```python
from build123d import *

# Parameters (mm, degrees)
BOSS_EXTRUDE1_DEPTH = 12


with BuildPart() as part:
    # Sketch1 → Boss-Extrude1 (new body)
    with BuildSketch(Plane.XY):
        with BuildLine():
            Line((140, 147), (378, 147))
            ThreePointArc((378, 147), (406.284271247, 135.284271247), (418, 107))
            Line((418, 107), (418, 0))
            Line((418, 0), (944.5, 0))
            Line((944.5, 0), (958.236494969, 111.874773736))
            ThreePointArc((958.236494969, 111.874773736), (971.433539106, 136.958228832), (997.938341035, 147))
            Line((997.938341035, 147), (1273.561658965, 147))
            ThreePointArc((1273.561658965, 147), (1300.066460894, 136.958228832), (1313.263505031, 111.874773736))
            Line((1313.263505031, 111.874773736), (1327, 0))
            Line((1327, 0), (1843, 0))
            Line((1843, 0), (1843, 107))
            ThreePointArc((1843, 107), (1854.715728753, 135.284271247), (1883, 147))
            Line((1883, 147), (2158, 147))
            ThreePointArc((2158, 147), (2186.284271247, 135.284271247), (2198, 107))
            Line((2198, 107), (2198, 0))
            Line((2198, 0), (2388, 0))
            Line((2388, 0), (2400, 12))
            Line((2400, 12), (2400, 195))
            Line((2400, 195), (2388, 207))
            Line((2388, 207), (12, 207))
            Line((12, 207), (0, 195))
            Line((0, 195), (0, 12))
            Line((0, 12), (12, 0))
            Line((12, 0), (100, 0))
            Line((100, 0), (100, 107))
            ThreePointArc((100, 107), (111.715728753, 135.284271247), (140, 147))
        make_face()
    extrude(amount=BOSS_EXTRUDE1_DEPTH)


solid = part.part
```
CAD build for the part. Positions are in the model's coordinates, mm. A direction names the side the tool comes from. Coordinates: 2 decimals unless noted, no trailing zeros. Loops run counter-clockwise (first coordinate to the right, second up) from the corner with the lowest first, then second, coordinate; pieces in that order, holes last. Notation, with made-up numbers: (23, -37) - (35, -37) arc R6 ccw to (35, -27) - close; hole circle Ø4 at (50.25, -37.5). An arc over 180 degrees is marked (long way). Use CSV: the item, a comma, the result in double quotes. Start each with the question number.
Q1. Drop flat-ended pins along their axis: P1, Ø3, axis at y = 185, z = 4.5, coming from the -X side; P2, Ø3, axis at x = 1288, z = 3.5, coming from the -Y side; P3, Ø6, axis at x = 2037.5, z = 8, coming from the -Y side. Give the stop position or say it passes through.
Q2. Probe probe 1 along X at (y, z) = (111, 4.75); probe 2 along X at (y, z) = (124.5, 3.75); probe 3 along Y at (x, z) = (1896, 11). List the from-to ranges inside material, lowest first. Write a range as from..to.
Q3. Cut at A-A, the plane y = 51. List the corners of the cut face in (x, z).
Q4. Two-plate mould, pull along X, no slides. Class faces 3 (the flat face through (1183, 151, 12)), 4 (the cylindrical face through (1854.406, 134.972, 5.916)): +X half, -X half, draft (parallel to the pull), parting line (faces both ways), or undercut.
Q5. Cut at C-C, the plane x = 270. List the corners of the cut face in (y, z).
Q6. Cut at B-B, the plane z = 2.75. List the corners of the cut face in (x, y).
Q7. 3-axis set-ups, long thin cutter, end or side, ignore diameter. For faces 1 (the flat face through (1183, 151, 0)), 2 (the cylindrical face through (405.972, 135.594, 5.916)): which of +Z, -Z, +X, -X, +Y, -Y reach the whole face in a straight line?
Here are the results:
1,P1,"x = 0"
1,P2,"y = 143.69"
1,P3,"y = 147"
2,probe 1,"0..100.2, 417.8..958.13, 1313.37..1843.2, 2197.8..2400"
2,probe 2,"0..104.03, 413.97..961.97, 1309.53..1847.03, 2193.97..2400"
2,probe 3,"147..207"
3,outline,"(0, 0) - (100, 0) - (100, 12) - (0, 12) - close; (418, 0) - (950.76, 0) - (950.76, 12) - (418, 12) - close; (1320.74, 0) - (1843, 0) - (1843, 12) - (1320.74, 12) - close; (2198, 0) - (2400, 0) - (2400, 12) - (2198, 12) - close"
4,face 3,"draft"
4,face 4,"undercut"
5,outline,"(147, 0) - (207, 0) - (207, 12) - (147, 12) - close"
6,outline,"(0, 12) - (12, 0) - (100, 0) - (100, 107) arc R40 cw to (140, 147) - (378, 147) arc R40 cw to (418, 107) - (418, 0) - (944.5, 0) - (958.24, 111.87) arc R40 cw to (997.94, 147) - (1273.56, 147) arc R40 cw to (1313.26, 111.87) - (1327, 0) - (1843, 0) - (1843, 107) arc R40 cw to (1883, 147) - (2158, 147) arc R40 cw to (2198, 107) - (2198, 0) - (2388, 0) - (2400, 12) - (2400, 195) - (2388, 207) - (12, 207) - (0, 195) - close"
7,face 1,"-Z, +X, -X, +Y, -Y"
7,face 2,"+Z, -Z, -Y"
